Build history of the part. All positions in model axes, mm. Face numbers are marked on the shaded views. Give positions to 0.01 mm unless a question says otherwise; leave off trailing zeros. Order: outer loops, then holes, each group sorted by start corner. A loop starts at its lowest first (then second) coordinate and runs counter-clockwise, first axis right, second up. Notation, with made-up numbers: (-7, 69) -> (37, 69) arc R22 ccw to (37, 78) -> close; hole circle Ø8 at (-13.75, 17.25). An arc over 180 degrees is marked (long way). One line per item, written item: value. Start each with the question number.
(1) Pin check, flat tips, straight feed: pin 1 (4 mm diameter, centred on x = 26.5, z = -15.5, fed in from +Y); pin 2 (6 mm diameter, centred on x = -24, y = 2.5, fed in from +Z); pin 3 (5 mm diameter, centred on x = 38.5, z = -2, fed in from +Y); pin 4 (25 mm diameter, centred on x = -6.5, z = -6.5, fed in from -Y). Stop position of each tip, or through.
(2) Probe line 1 (Y direction, x = 43.5, z = -8); line 2 (Z direction, x = -41, y = 9); line 3 (Y direction, x = -43.5, z = -5). List the from-to ranges inside material, lowest first.
(3) Two-plate mould, pull along X, no slides. Class the marked faces 1, 2, 3 and 4: +X half, -X half, draft (parallel to the pull), parting line (faces both ways), or undercut.
(4) Saw through at B-B on z = 42.5. Give the cut face in (x, y).
(5) Saw through at A-A on x = 38. Give the cut face in (y, z).
```python
from build123d import *
from build123d.topology import SkipClean

# Parameters (mm, degrees)
BASE_PLATE_DEPTH          = 3
MOUNTING_EARS_DEPTH       = 7
BEARING_HUB_DEPTH         = 13
COUNTERBORE_SKETCH_R      = 8
COUNTERBORES_2X_16_DEPTH  = 5
MOUNTING_HOLE_SKETCH_R    = 4.5
MOUNTING_HOLES_2X_9_DEPTH = 5


with BuildPart() as part:
    # Base Plate Sketch → Base Plate (new body)
    with BuildSketch(Plane(origin=(0, 0, 0), x_dir=(1, 0, 0), z_dir=(0, 1, 0))):
        with BuildLine():
            Line((-42.105263158, 11.275939624), (-8.552631579, 23.491540883))
            ThreePointArc((-8.552631579, 23.491540883), (0, 25), (8.552631579, 23.491540883))
            Line((8.552631579, 23.491540883), (42.105263158, 11.275939624))
            ThreePointArc((42.105263158, 11.275939624), (49.60820541, 3.041310105), (47.10686849, -7.814406331))
            Line((47.10686849, -7.814406331), (15.178114149, -45.024010552))
            ThreePointArc((15.178114149, -45.024010552), (0, -52), (-15.178114149, -45.024010552))
            Line((-15.178114149, -45.024010552), (-47.10686849, -7.814406331))
            ThreePointArc((-47.10686849, -7.814406331), (-49.60820541, 3.041310105), (-42.105263158, 11.275939624))
        make_face()
    extrude(amount=BASE_PLATE_DEPTH)

    # Ear and Hub Profile Sketch → Mounting Ears (add)
    with BuildSketch(Plane(origin=(0, 3, 0), x_dir=(1, 0, 0), z_dir=(0, 1, 0))):
        with BuildLine():
            ThreePointArc((-26, 0), (-31.117527984, -9.830136263), (-42.105263158, -11.275939624))
            Line((-42.105263158, -11.275939624), (-8.552631579, -23.491540883))
            ThreePointArc((-8.552631579, -23.491540883), (-25, 0), (-8.552631579, 23.491540883))
            Line((-8.552631579, 23.491540883), (-42.105263158, 11.275939624))
            ThreePointArc((-42.105263158, 11.275939624), (-31.117527984, 9.830136263), (-26, 0))
        make_face()
        with BuildLine():
            ThreePointArc((-47.10686849, -7.814406331), (-44.829030594, -9.867337085), (-42.105263158, -11.275939624))
            ThreePointArc((-42.105263158, -11.275939624), (-31.117527984, -9.830136263), (-26, 0))
            ThreePointArc((-26, 0), (-31.117527984, 9.830136263), (-42.105263158, 11.275939624))
            ThreePointArc((-42.105263158, 11.275939624), (-49.60820541, 3.041310105), (-47.10686849, -7.814406331))
        make_face()
        with BuildLine():
            ThreePointArc((25, 0), (20.479450548, -14.338483367), (8.552631579, -23.491540883))
            Line((8.552631579, -23.491540883), (42.105263158, -11.275939624))
            ThreePointArc((42.105263158, -11.275939624), (26, 0), (42.105263158, 11.275939624))
            Line((42.105263158, 11.275939624), (8.552631579, 23.491540883))
            ThreePointArc((8.552631579, 23.491540883), (20.479450548, 14.338483367), (25, 0))
        make_face()
        with BuildLine():
            ThreePointArc((42.105263158, 11.275939624), (26, 0), (42.105263158, -11.275939624))
            ThreePointArc((42.105263158, -11.275939624), (44.829030594, -9.867337085), (47.10686849, -7.814406331))
            ThreePointArc((47.10686849, -7.814406331), (49.25349772, -4.166388011), (50, 0))
            ThreePointArc((50, 0), (47.830136263, 6.882472016), (42.105263158, 11.275939624))
        make_face()
    extrude(amount=MOUNTING_EARS_DEPTH)

    # Sketch2_5 → Bearing Hub (add)
    with SkipClean():  # the faces are left unmerged after this step: merging them gives an invalid solid
        with BuildSketch(Plane(origin=(0, 3, 0), x_dir=(1, 0, 0), z_dir=(0, 1, 0))):
            with BuildLine():
                ThreePointArc((-8.552631579, 23.491540883), (-25, 0), (-8.552631579, -23.491540883))
                ThreePointArc((-8.552631579, -23.491540883), (0, -25), (8.552631579, -23.491540883))
                ThreePointArc((8.552631579, -23.491540883), (20.479450548, -14.338483367), (25, 0))
                ThreePointArc((25, 0), (20.479450548, 14.338483367), (8.552631579, 23.491540883))
                ThreePointArc((8.552631579, 23.491540883), (0, 25), (-8.552631579, 23.491540883))
            make_face()
        extrude(amount=BEARING_HUB_DEPTH)

    # Bearing Bore Profile Sketch → Bearing Bore (revolve, cut)
    with SkipClean():  # the faces are left unmerged after this step: merging them gives an invalid solid
        with BuildSketch(Plane.XY, mode=Mode.PRIVATE) as bearing_bore_sk:
            Polygon((21.083967654, 16), (0, 16), (0, 0), (14, 0), (14, 1.5), (15.5, 1.5), (15.5, 3), (14, 3), (14, 6.25), (15.5, 6.25), (15.5, 7.75), (14, 7.75), (14, 11), (15.5, 11), (15.5, 12.5), (14, 12.5), (14, 14), (19.083967654, 14), align=None)
        revolve(bearing_bore_sk.sketch.rotate(Axis((0, 16, 0), (0, -1, 0)), 90), axis=Axis((0, 16, 0), (0, -1, 0)), mode=Mode.SUBTRACT)

    # Counterbore Sketch → Counterbores 2x_16 (cut)
    with SkipClean():  # the faces are left unmerged after this step: merging them gives an invalid solid
        with BuildSketch(Plane(origin=(0, 10, 0), x_dir=(1, 0, 0), z_dir=(0, 1, 0))):
            with Locations(Location((38, 0, 0), (0, 0, 270))):
                Circle(COUNTERBORE_SKETCH_R)
            with Locations(Location((-38, 0, 0), (0, 0, 270))):
                Circle(COUNTERBORE_SKETCH_R)
        extrude(amount=-COUNTERBORES_2X_16_DEPTH, mode=Mode.SUBTRACT)

    # Mounting Hole Sketch → Mounting Holes 2x_9 (cut)
    with SkipClean():  # the faces are left unmerged after this step: merging them gives an invalid solid
        with BuildSketch(Plane(origin=(0, 5, 0), x_dir=(1, 0, 0), z_dir=(0, 1, 0))):
            with Locations(Location((38, 0, 0), (0, 0, 270))):
                Circle(MOUNTING_HOLE_SKETCH_R)
            with Locations(Location((-38, 0, 0), (0, 0, 270))):
                Circle(MOUNTING_HOLE_SKETCH_R)
        extrude(amount=-MOUNTING_HOLES_2X_9_DEPTH, mode=Mode.SUBTRACT)


solid = part.part
```
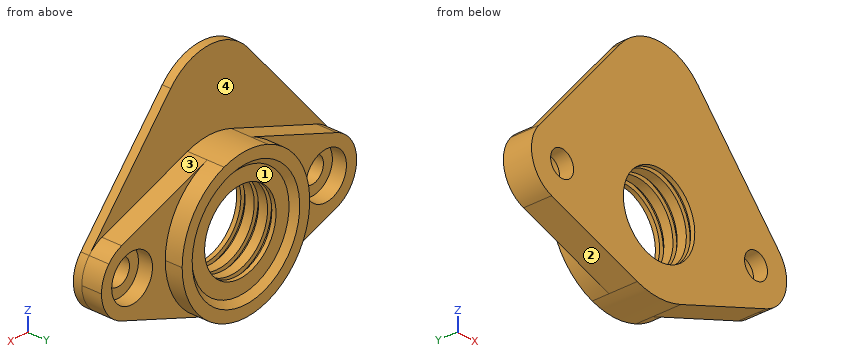
Results below:
1. pin 1: stops at y = 10
1. pin 2: stops at z = 38.24
1. pin 3: stops at y = 5
1. pin 4: stops at y = 0
2. line 1: y = 0 to 10
2. line 2: z = -11.68 to -7.42, 7.42 to 11.68
2. line 3: y = 0 to 5
3. face 1: undercut
3. face 2: -X half
3. face 3: +X half
3. face 4: draft
4. outline: (-17.34, 0) -> (17.34, 0) -> (17.34, 3) -> (-17.34, 3) -> close
5. outline: (0, -12.77) -> (10, -12.77) -> (10, -8) -> (5, -8) -> (5, -4.5) -> (0, -4.5) -> close; (0, 4.5) -> (5, 4.5) -> (5, 8) -> (10, 8) -> (10, 12.77) -> (3, 12.77) -> (3, 18.43) -> (0, 18.43) -> close
